```python
from build123d import *

# Parameters (mm, degrees)
SKETCH1_W                  = 180
SKETCH1_H                  = 40
BOSS_EXTRUDE1_DEPTH        = 5
F_13_0_13_DIAMETER_HOLE1_D = 13


with BuildPart() as part:
    # Sketch1 → Boss-Extrude1 (new, symmetric)
    with BuildSketch(Plane.XY):
        Rectangle(SKETCH1_W, SKETCH1_H)
    extrude(amount=BOSS_EXTRUDE1_DEPTH, both=True)

    # Ø13.0 (13) Diameter Hole1 (through all)
    with Locations(Plane.XY.offset(5)):
        with Locations((-70, 0), (70, 0)):
            Hole(F_13_0_13_DIAMETER_HOLE1_D / 2)


solid = part.part
```
Geometry check sheet. Reference: the model listing, model coordinates, mm. Round coordinates to 2 decimals unless told otherwise and drop trailing zeros. Order: outer loops, then holes, each group sorted by start corner. A loop starts at its lowest first (then second) coordinate and runs counter-clockwise, first axis right, second up. Notation, with made-up numbers: (87, 30) - (96, 30) arc R26 ccw to (96, 52) - close; hole circle Ø5 at (86.5, 34.5). An arc over 180 degrees is marked (long way). Use a Markdown table: item, result. Add a question column.
1) Section check C-C (z = -1.5). Record the cut outline in (x, y).
2) Section check B-B (x = -70). Record the cut outline in (y, z), then the cut area to 3 significant figures.
3) Section check A-A (y = 0). Record the cut outline in (x, z).
4) Thickness scan on line 1 along Y through (x, z) = (70, -0.25); line 2 along X through (y, z) = (3, 1.75); line 3 along X through (y, z) = (-1, 4). Record the ranges inside material, lowest first.
5) Mould release check, pull along X, two halves, no side actions. Record for faces 1 (the cylindrical face through (-76, -2.5, -0.1)), 2 (the flat face through (-90, 0, 0)), 3 (the flat face through (-1, -20, 0)): released by +X, released by -X, zero draft, split by the parting line, or undercut.
Established:
| question | item | result |
|---|---|---|
| 1 | outline | (-90, -20) - (90, -20) - (90, 20) - (-90, 20) - close; hole circle Ø13 at (-70, 0); hole circle Ø13 at (70, 0) |
| 2 | outline | (-20, -5) - (-6.5, -5) - (-6.5, 5) - (-20, 5) - close; (6.5, -5) - (20, -5) - (20, 5) - (6.5, 5) - close |
| 2 | area | 270 mm2 |
| 3 | outline | (-90, -5) - (-76.5, -5) - (-76.5, 5) - (-90, 5) - close; (-63.5, -5) - (63.5, -5) - (63.5, 5) - (-63.5, 5) - close; (76.5, -5) - (90, -5) - (90, 5) - (76.5, 5) - close |
| 4 | line 1 | -20 to -6.5, 6.5 to 20 |
| 4 | line 2 | -90 to -75.77, -64.23 to 64.23, 75.77 to 90 |
| 4 | line 3 | -90 to -76.42, -63.58 to 63.58, 76.42 to 90 |
| 5 | face 1 | undercut |
| 5 | face 2 | released by -X |
| 5 | face 3 | zero draft |
